Model file for the job. Use its own axes, mm. A direction names the side the tool comes from. Coordinates: 2 decimals unless noted, no trailing zeros. Loops run counter-clockwise (first coordinate to the right, second up) from the corner with the lowest first, then second, coordinate; pieces in that order, holes last. Notation, with made-up numbers: M 33,64 L 55,64 A9 cw 55,71 Z; hole C 22.25,6 d7. An arc over 180 degrees is marked long. One line per question, with ' | ' between items. Start each with the question number.
```python
from build123d import *

# Parameters (mm, degrees)
SKETCH_1_W          = 6.99
SKETCH_1_H          = 21
SKETCH_4_R          = 8
CUT_EXTRUDE_3_DEPTH = 5
SKETCH_5_R          = 15
SKETCH_5_R_2        = 8
EXTRUDE_1_DEPTH     = 2
CHAMFER_1_SIZE      = 1
CHAMFER_1_SIZE2     = 0.577350269
CHAMFER_2_SIZE      = 1
CHAMFER_2_SIZE2     = 0.577350269


with BuildPart() as part:
    # 草图1 → 旋转1 (revolve)
    with BuildSketch(Plane.XY, mode=Mode.PRIVATE) as revolve_1_sk:
        with Locations((9.495, 0)):
            Rectangle(SKETCH_1_W, SKETCH_1_H)
    revolve(revolve_1_sk.sketch.rotate(Axis((0, 0, 0), (0, 1, 0)), 90), axis=Axis((0, 0, 0), (0, 1, 0)))

    # 草图4 → 切除-拉伸3 (cut)
    with BuildSketch(Plane.XZ.offset(10.5)):
        with Locations(Location((0, 0, 0), (0, 0, 270))):
            Circle(SKETCH_4_R)
    cut_extrude_3 = extrude(amount=-CUT_EXTRUDE_3_DEPTH, mode=Mode.SUBTRACT)

    # 草图5 → 凸台-拉伸1 (add)
    with BuildSketch(Plane.XZ.offset(10.5)):
        with Locations(Location((0, 0, 0), (0, 0, 270))):
            Circle(SKETCH_5_R)
        with Locations(Location((0, 0, 0), (0, 0, 270))):
            Circle(SKETCH_5_R_2, mode=Mode.SUBTRACT)
    extrude_1 = extrude(amount=-EXTRUDE_1_DEPTH)

    # 镜向1: 切除-拉伸3, 凸台-拉伸1 across plane
    add(cut_extrude_3.mirror(Plane.ZX), mode=Mode.SUBTRACT)
    add(extrude_1.mirror(Plane.ZX))

    # 倒角1
    chamfer_1_edges = [part.edges().sort_by_distance(p)[0] for p in [
        (0, 8.5, 15),
    ]]
    chamfer_1_side = [part.faces().sort_by_distance(p)[0] for p in [
        (0, 9.5, 15),
    ]]
    chamfer(chamfer_1_edges, length=CHAMFER_1_SIZE, length2=CHAMFER_1_SIZE2, reference=chamfer_1_side[0])

    # 倒角2
    chamfer_2_edges = [part.edges().sort_by_distance(p)[0] for p in [
        (0, -8.5, 15),
    ]]
    chamfer_2_side = [part.faces().sort_by_distance(p)[0] for p in [
        (0, -8.5, 14.575735931),
    ]]
    chamfer(chamfer_2_edges, length=CHAMFER_2_SIZE, length2=CHAMFER_2_SIZE2, reference=chamfer_2_side[0])


solid = part.part
```
(1) Band-saw the part on A-A on z = 0. Write the cut outline in (x, y), then the cut area to 3 significant figures.
(2) 3-axis set-ups, long thin cutter, end or side, ignore diameter. For faces 5 (the face through (-6, -10.5, -6)), 6 (the face through (-0.571, 0.119, 12.977)), 7 (the face through (6, -5.5, 2)): which of +Z, -Z, +X, -X, +Y, -Y reach the whole face in a straight line?
(3) Band-saw the part on C-C on y = 1. Write the cut outline in (x, z), then the cut area to 3 significant figures.
(4) Band-saw the part on B-B on x = 0. Write the cut outline in (y, z), then the cut area to 3 significant figures.
(5) Two-plate mould, pull along Z, no slides. Class faces 1 (the face through (0.66, 10.007, 14.985)), 2 (the face through (-7.81, 8.04, 1.73)), 3 (the face through (6, 5.5, 2)), 4 (the face through (2, 8.5, 13)): pulls with the +Z half, pulls with the -Z half, needs draft (parallel to the pull), parting line crosses it, or undercut.
(6) Drill centre lines: line 1 (X direction, y = 0, z = 0); line 2 (X direction, y = -9.1, z = 0); line 3 (Y direction, x = -5.5, z = 12.25). Where is each one in solid material? Low to high. Write a range as [from, to].
(7) Band-saw the part on D-D on y = 7.25. Write the cut outline in (x, z), then the cut area to 3 significant figures.
(8) Pin check, flat tips, straight feed: P1, Ø6, axis at y = 7, z = -3.5, coming from the +X side; P2, Ø1, axis at x = -11, y = 2.5, coming from the -Z side; P3, Ø4, axis at x = -4.5, y = 3.5, coming from the -Z side. Stop position of each tip, or through.
Computed values:
1) outline: M -15,-10.5 L -8,-10.5 L -8,-5.5 L -6,-5.5 L -6,5.5 L -8,5.5 L -8,10.5 L -15,10.5 L -15,9.5 L -14.42,8.5 L -12.99,8.5 L -12.99,-8.5 L -14,-8.5 L -15,-9.08 Z; M 6,-5.5 L 8,-5.5 L 8,-10.5 L 15,-10.5 L 15,-9.08 L 14,-8.5 L 12.99,-8.5 L 12.99,8.5 L 14.42,8.5 L 15,9.5 L 15,10.5 L 8,10.5 L 8,5.5 L 6,5.5 Z | area: 269 mm^2
2) face 5: +Z, -Z, +X, -X, -Y | face 6: none | face 7: -Y
3) outline: C 0,0 d25.98; hole C 0,0 d12 | area: 417 mm^2
4) outline: M -10.5,-15 L -9.08,-15 L -8.5,-14 L -8.5,-12.99 L 8.5,-12.99 L 8.5,-14.42 L 9.5,-15 L 10.5,-15 L 10.5,-8 L 5.5,-8 L 5.5,-6 L -5.5,-6 L -5.5,-8 L -10.5,-8 Z; M -10.5,8 L -5.5,8 L -5.5,6 L 5.5,6 L 5.5,8 L 10.5,8 L 10.5,15 L 9.5,15 L 8.5,14.42 L 8.5,12.99 L -8.5,12.99 L -8.5,14 L -9.08,15 L -10.5,15 Z | area: 269 mm^2
5) face 1: parting line crosses it | face 2: undercut | face 3: undercut | face 4: needs draft
6) line 1: [-12.99, -6], [6, 12.99] | line 2: [-15, -8], [8, 15] | line 3: [-10.5, -8.5], [8.5, 10.5]
7) outline: C 0,0 d25.98; hole C 0,0 d16 | area: 329 mm^2
8) P1: x = 14.89 | P2: z = -7.65 | P3: z = -12.75
